Work out the finished part from the listing and answer in its coordinate system (mm). Face numbers are marked on the shaded views. A direction names the side the tool comes from. Give positions to 0.01 mm unless a question says otherwise; leave off trailing zeros. Loops run counter-clockwise (first coordinate to the right, second up) from the corner with the lowest first, then second, coordinate; pieces in that order, holes last.
```python
from build123d import *

# Parameters (mm, degrees)
SKETCH_1_W                = 45
SKETCH_1_H                = 10
EXTRUDE_1_DEPTH           = 8
HOLE_WIZARD_1_D           = 3.2
HOLE_WIZARD_1_CBORE_D     = 6
HOLE_WIZARD_1_CBORE_DEPTH = 3.5
SKETCH_4_W                = 45
SKETCH_4_H                = 8
EXTRUDE_2_DEPTH           = 5


with BuildPart() as part:
    # 草图1 → 凸台-拉伸1 (new body)
    with BuildSketch(Plane(origin=(0, 0, 0), x_dir=(1, 0, 0), z_dir=(0, 1, 0))):
        Rectangle(SKETCH_1_W, SKETCH_1_H)
    extrude(amount=EXTRUDE_1_DEPTH)

    # 打孔尺寸(%根据)开槽圆柱头螺钉的类型1 (through all)
    with Locations(Plane(origin=(0, 8, 0), x_dir=(1, 0, 0), z_dir=(0, 1, 0))):
        with Locations((-7.5, 0), (7.5, 0)):
            CounterBoreHole(HOLE_WIZARD_1_D / 2, HOLE_WIZARD_1_CBORE_D / 2, HOLE_WIZARD_1_CBORE_DEPTH)

    # 草图4 → 凸台-拉伸2 (add)
    with BuildSketch(Plane.XY.offset(5)):
        with Locations((0, 4)):
            Rectangle(SKETCH_4_W, SKETCH_4_H)
    extrude(amount=EXTRUDE_2_DEPTH)


solid = part.part
```
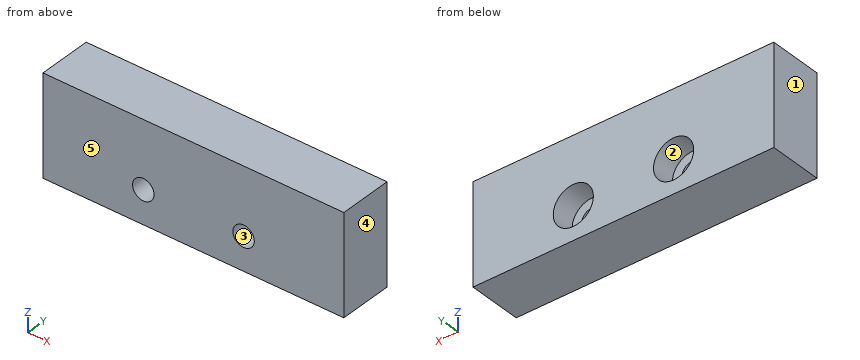
Q1. Given pin 1 (5.5 mm diameter, centred on x = 7.5, z = 0, fed in from +Y), flat-ended and moving along its own axis, determine where the tip first touches the part or whether it passes through.
Q2. Section D-D on x = 6.5 is taken. Give the vertices of the cut face in (y, z).
Q3. Consider line 1 along Z through (x, y) = (7.5, 6.4); line 2 along X through (y, z) = (5.5, -2.5); line 3 along Z through (x, y) = (7.5, 1.15). Determine where each line is inside the solid, lowest interval first.
Q4. Determine the mould class of the marked faces 3, 4 and 5 for opening direction X: +X half, -X half, draft (parallel to the pull), parting line (faces both ways), or undercut.
Q5. Which of the six approach directions +Z, -Z, +X, -X, +Y, -Y give full straight-line access (tool end or side, diameter ignored) to the marked faces 1 and 2?
Q6. Section B-B on y = 7 is taken. Give the vertices of the cut face in (x, z).
Q7. Section C-C on y = 3.75 is taken. Give the vertices of the cut face in (x, z).
Q8. Section A-A on x = -7.5 is taken. Give the vertices of the cut face in (y, z).
Check result:
1. pin 1: stops at y = 4.5
2. outline: (0, -5) - (8, -5) - (8, -2.83) - (4.5, -2.83) - (4.5, -1.25) - (0, -1.25) - close; (0, 1.25) - (4.5, 1.25) - (4.5, 2.83) - (8, 2.83) - (8, 10) - (0, 10) - close
3. line 1: z = -5 to -3, 3 to 10
3. line 2: x = -22.5 to -9.16, -5.84 to 5.84, 9.16 to 22.5
3. line 3: z = -5 to -1.6, 1.6 to 10
4. face 3: undercut
4. face 4: +X half
4. face 5: draft
5. face 1: +Z, -Z, -X, +Y, -Y
5. face 2: +Y
6. outline: (-22.5, -5) - (22.5, -5) - (22.5, 10) - (-22.5, 10) - close; hole circle Ø6 at (-7.5, 0); hole circle Ø6 at (7.5, 0)
7. outline: (-22.5, -5) - (22.5, -5) - (22.5, 10) - (-22.5, 10) - close; hole circle Ø3.2 at (-7.5, 0); hole circle Ø3.2 at (7.5, 0)
8. outline: (0, -5) - (8, -5) - (8, -3) - (4.5, -3) - (4.5, -1.6) - (0, -1.6) - close; (0, 1.6) - (4.5, 1.6) - (4.5, 3) - (8, 3) - (8, 10) - (0, 10) - close
